```python
from build123d import *

# Parameters (mm, degrees)
SKETCH_1_R              = 25
EXTRUDE_1_DEPTH         = 710
SKETCH_2_R              = 20
EXTRUDE_2_DEPTH         = 95
SKETCH_3_R              = 18
EXTRUDE_3_DEPTH         = 30
HOLE_WIZARD_M12_1_D     = 10.2
HOLE_WIZARD_M12_1_DEPTH = 32.75
HOLE_WIZARD_M12_1_TIP   = 3.064389157
SKETCH_8_R              = 20
SKETCH_8_R_2            = 16
CUT_EXTRUDE_1_DEPTH     = 2


with BuildPart() as part:
    # 草图1 → 拉伸1 (new body)
    with BuildSketch(Plane.XY):
        Circle(SKETCH_1_R)
    extrude(amount=EXTRUDE_1_DEPTH)

    # 草图2 → 拉伸2 (add)
    with BuildSketch(Plane.XY.offset(710)):
        Circle(SKETCH_2_R)
    extrude(amount=EXTRUDE_2_DEPTH)

    # 草图3 → 拉伸3 (add)
    with BuildSketch(Plane.XY.offset(805)):
        Circle(SKETCH_3_R)
    extrude(amount=EXTRUDE_3_DEPTH)

    # M12 螺纹孔1
    with Locations(Plane(origin=(0, 0, 0), x_dir=(-1, 0, 0), z_dir=(0, 0, -1))):
        with Locations((0, 0)):
            Hole(HOLE_WIZARD_M12_1_D / 2, depth=HOLE_WIZARD_M12_1_DEPTH)
            with Locations((0, 0, -(HOLE_WIZARD_M12_1_DEPTH + HOLE_WIZARD_M12_1_TIP / 2))):  # 118° drill point
                Cone(0, HOLE_WIZARD_M12_1_D / 2, HOLE_WIZARD_M12_1_TIP, mode=Mode.SUBTRACT)

    # 草图7 → 切除-旋转1 (revolve, cut)
    with BuildSketch(Plane(origin=(0, 0, 0), x_dir=(1, 0, 0), z_dir=(0, 1, 0))):
        Polygon((-2, -835), (0, -833), (0, -835), align=None)
    revolve(axis=Axis((0, 0, 835), (0, 0, -1)), mode=Mode.SUBTRACT)

    # 草图8 → 切除-拉伸1 (cut)
    with BuildSketch(Plane.XY.offset(805)):
        Circle(SKETCH_8_R)
        Circle(SKETCH_8_R_2, mode=Mode.SUBTRACT)
    extrude(amount=CUT_EXTRUDE_1_DEPTH, mode=Mode.SUBTRACT)


solid = part.part
```
Model file for the job. Use its own axes, mm. A direction names the side the tool comes from. Give positions to 0.01 mm unless a question says otherwise; leave off trailing zeros. Loops run counter-clockwise (first coordinate to the right, second up) from the corner with the lowest first, then second, coordinate; pieces in that order, holes last. Notation, with made-up numbers: (-34, -26) - (4, -26) arc R21 cw to (4, -14) - close; hole circle Ø11 at (13.5, 69.5). An arc over 180 degrees is marked (long way). One line per item, written item: value. Start each with the question number.
1. Probe L1, parallel to Z at x = 13, y = 10; L2, parallel to Y at x = 15, z = 192. List the from-to ranges inside material, lowest first. Write a range as from..to.
2. Pull direction Z, two halves, no side cores. Call faces 4 (the cylindrical face through (-2.343, 17.847, 820.804)), 5 (the flat face through (0, -4, 835)), 6 (the flat face through (-8.98, 13.43, 805)): pulls with the +Z half, pulls with the -Z half, needs draft (parallel to the pull), parting line crosses it, or undercut.
3. Pin check, flat tips, straight feed: pin 1 (1.5 mm diameter, centred on y = -13, z = 559, fed in from -X); pin 2 (3 mm diameter, centred on x = 13, z = 573.5, fed in from +Y); pin 3 (2 mm diameter, centred on x = -13.5, y = -19, fed in from +Z). Stop position of each tip, or through.
4. Which spindle directions (+Z, -Z, +X, -X, +Y, -Y) get a long thin tool onto all of the face, cutting with end or side? Do faces 1 (the cylindrical face through (-3.47, -15.62, 805.99)), 2 (the cylindrical face through (-4.336, -19.524, 756.835)), 3 (the cylindrical face through (23.846, 7.509, 350.03)). Say none if no direction does.
5. Slice it at A-A (z = 189). List the corners of the cut face in (x, y).
Solution:
1. L1: z = 0..805, 807..835
1. L2: y = -20..20
2. face 4: needs draft
2. face 5: pulls with the +Z half
2. face 6: undercut
3. pin 1: stops at x = -21.79
3. pin 2: stops at y = 22.2
3. pin 3: stops at z = 710
4. face 1: none
4. face 2: +Z
4. face 3: +Z, -Z
5. outline: circle Ø50 at (0, 0)
